Input: dimensioned drawing with shaded views. Units: mm. Origin: part minimum x, y, z. A direction names the side the tool comes from. Give positions to 0.01 mm unless a question says otherwise; leave off trailing zeros. Loops run counter-clockwise (first coordinate to the right, second up) from the corner with the lowest first, then second, coordinate; pieces in that order, holes last. Notation, with made-up numbers: M -38,15 L 14,15 A23 cw 14,43 Z; hole C -2,67.5 d11. An arc over 180 degrees is marked long. Use CSV: the item, a comma, the result in double quotes. Start each with the question number.
Q1. Section A-A, the plane y = 69. Output: boundary loops of the cut face in (x, z).
Q2. Section C-C, the plane x = 16. Output: boundary loops of the cut face in (y, z).
Q3. Section B-B, the plane y = 5. Output: boundary loops of the cut face in (x, z), plus the area to 4 significant figures.
Q4. Pin query (flat end, axial travel): pin 1 (7 mm diameter, centred on x = 21, y = 5, fed in from -Z); pin 2 (4 mm diameter, centred on x = 22, z = 10.5, fed in from -Y); pin 3 (12 mm diameter, centred on x = 11, z = 18.5, fed in from +Y). Return the tip coordinate at first contact, or that it passes through.
Q5. Material intervals for line 1 along Y through (x, z) = (6, 17.05); line 2 along X through (y, z) = (7, 17); line 3 along X through (y, z) = (15.5, 18.5), sorted ascending.
Q6. Section D-D, the plane y = 42. Output: boundary loops of the cut face in (x, z).
Q7. Reachability of the marked faces 1, 2, 3 and 4 from +Z, -Z, +X, -X, +Y, -Y: full face, straight path, thin tool, end or side. Return the list, or none.
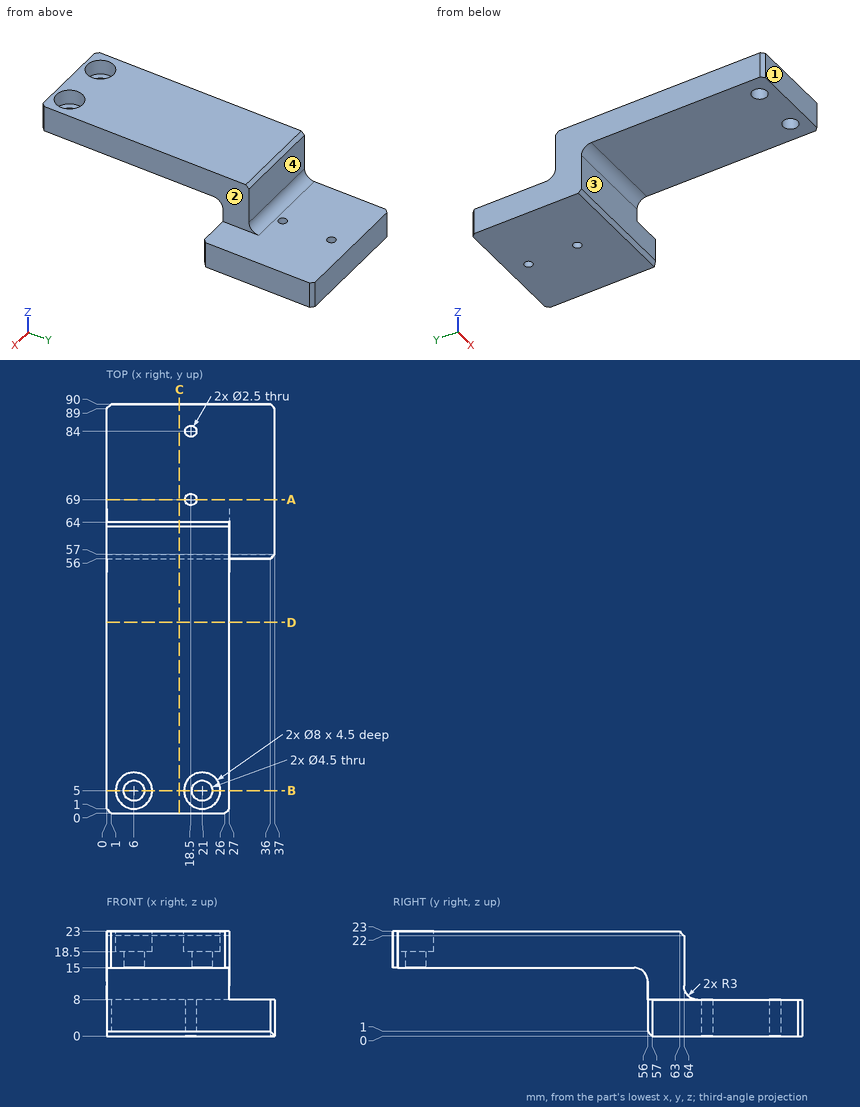
A:
1,outline,"M 0,0 L 17.25,0 L 17.25,8 L 0,8 Z; M 19.75,0 L 37,0 L 37,8 L 19.75,8 Z"
2,outline,"M 0,15 L 53,15 A3 cw 56,12 L 56,1 L 57,0 L 90,0 L 90,8 L 67,8 A3 cw 64,11 L 64,22 L 63,23 L 0,23 Z"
3,outline,"M 0,15 L 3.75,15 L 3.75,18.5 L 2,18.5 L 2,23 L 0,23 Z; M 8.25,15 L 18.75,15 L 18.75,18.5 L 17,18.5 L 17,23 L 10,23 L 10,18.5 L 8.25,18.5 Z; M 23.25,15 L 27,15 L 27,23 L 25,23 L 25,18.5 L 23.25,18.5 Z"
3,area,"112.5 mm^2"
4,pin 1,"z = 15"
4,pin 2,"y = 55.96"
4,pin 3,"y = 64"
5,line 1,"0 to 2.75, 7.25 to 64"
5,line 2,"0 to 4.97, 7.03 to 19.97, 22.03 to 27"
5,line 3,"0 to 27"
6,outline,"M 0,15 L 27,15 L 27,23 L 0,23 Z"
7,face 1,"+Z, -Z, +X, -X, -Y"
7,face 2,"+Z, +X, +Y, -Y"
7,face 3,"-Z, +X, -X, -Y"
7,face 4,"+Z, +X, -X, +Y"
